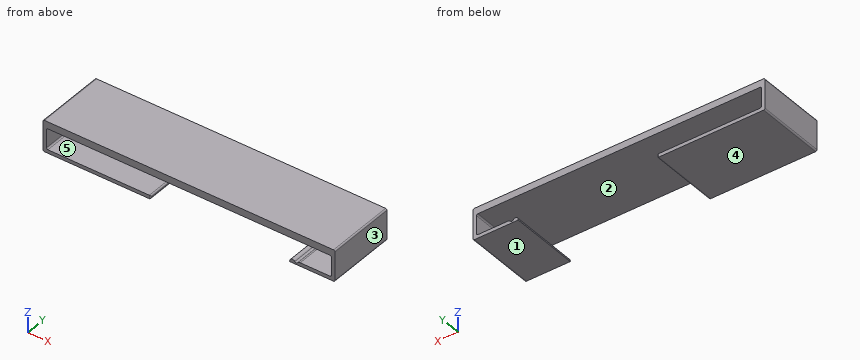
```python
from build123d import *

# Parameters (mm, degrees)
SKETCH1_W           = 15.5
SKETCH1_H           = 10
BOSS_EXTRUDE1_DEPTH = 0.5
SKETCH2_W           = 0.5
SKETCH2_H           = 10
BOSS_EXTRUDE2_DEPTH = 3
SKETCH3_W           = 42
SKETCH3_H           = 10
BOSS_EXTRUDE3_DEPTH = 1
SKETCH4_W           = 0.5
SKETCH4_H           = 10
BOSS_EXTRUDE4_DEPTH = 4.5
BOSS_EXTRUDE5_DEPTH = 10
FILLET1_R           = 0.2


with BuildPart() as part:
    # Sketch1 → Boss-Extrude1 (new body)
    with BuildSketch(Plane.XY):
        with Locations((-134.781169153, 115.619026916)):
            Rectangle(SKETCH1_W, SKETCH1_H)
    extrude(amount=BOSS_EXTRUDE1_DEPTH)

    # Sketch2 → Boss-Extrude2 (add)
    with BuildSketch(Plane.XY.offset(0.5)):
        with Locations((-142.281169153, 115.619026916)):
            Rectangle(SKETCH2_W, SKETCH2_H)
    extrude(amount=BOSS_EXTRUDE2_DEPTH)

    # Sketch3 → Boss-Extrude3 (add)
    with BuildSketch(Plane.XY.offset(3.5)):
        with Locations((-121.531169153, 115.619026916)):
            Rectangle(SKETCH3_W, SKETCH3_H)
    extrude(amount=BOSS_EXTRUDE3_DEPTH)

    # Sketch4 → Boss-Extrude4 (add)
    with BuildSketch(Plane.XY.offset(4.5)):
        with Locations((-100.781169153, 115.619026916)):
            Rectangle(SKETCH4_W, SKETCH4_H)
    extrude(amount=-BOSS_EXTRUDE4_DEPTH)

    # Sketch6 → Boss-Extrude5 (add)
    with BuildSketch(Plane(origin=(0, 110.619026916, 0), x_dir=(-1, 0, 0), z_dir=(0, -1, 0))):
        with BuildLine():
            Line((100.531169153, 0), (107.031169153, 0))
            Line((107.031169153, 0), (107.031169153, -0.1))
            ThreePointArc((107.031169153, -0.1), (106.754872908, -0.48039109), (106.307682248, -0.335279031))
            ThreePointArc((106.307682248, -0.335279031), (106.114215823, -0.2324803), (105.914058339, -0.321552283))
            ThreePointArc((105.914058339, -0.321552283), (105.742384515, -0.453197607), (105.531169153, -0.5))
            Line((105.531169153, -0.5), (100.531169153, -0.5))
            Line((100.531169153, -0.5), (100.531169153, 0))
        make_face()
    extrude(amount=-BOSS_EXTRUDE5_DEPTH)

    # Fillet1
    fillet1_edges = [part.edges().sort_by_distance(p)[0] for p in [
        (-127.031169153, 115.619026916, 0.5),
        (-142.031169153, 115.619026916, 0.5),
        (-142.031169153, 115.619026916, 3.5),
        (-142.531169153, 115.619026916, 4.5),
        (-100.531169153, 115.619026916, 4.5),
        (-100.531169153, 115.619026916, 0),
        (-101.031169153, 115.619026916, 3.5),
        (-127.031169153, 115.619026916, 0),
        (-142.531169153, 115.619026916, 0),
        (-101.031169153, 115.619026916, 0.5),
        (-127.031169153, 120.619026916, 0.25),
        (-127.031169153, 110.619026916, 0.25),
    ]]
    fillet(fillet1_edges, radius=FILLET1_R)


solid = part.part
```
Could you check a few things on this model? Use its own coordinates, in mm. Face numbers are marked on the shaded views. A direction names the side the tool comes from. Round coordinates to 2 decimals unless told otherwise and drop trailing zeros. Loops run counter-clockwise (first coordinate to the right, second up) from the corner with the lowest first, then second, coordinate; pieces in that order, holes last. Notation, with made-up numbers: (50, -32.75) - (92, -32.75) arc R34 ccw to (92, 6.25) - close; hole circle Ø10 at (58, 66.5). An arc over 180 degrees is marked (long way). Use CSV: the item, a comma, the result in double quotes.
Item 1: If we section it at B-B on x = -137: List the corners of the cut face in (y, z) for me.
Here are the results:
outline,"(110.62, 0) - (120.62, 0) - (120.62, 0.5) - (110.62, 0.5) - close; (110.62, 3.5) - (120.62, 3.5) - (120.62, 4.5) - (110.62, 4.5) - close"
Item 2: If we section it at D-D on x = -118: List the corners of the cut face in (y, z) for me.
Here are the results:
outline,"(110.62, 3.5) - (120.62, 3.5) - (120.62, 4.5) - (110.62, 4.5) - close"
Item 3: If we mould it in two halves opening along Z, with no side actions, what happens to the marked faces 3, 4 and 5? For each: pulls with the +Z half, pulls with the -Z half, needs draft (parallel to the pull), parting line crosses it, or undercut.
Here are the results:
face 3,"needs draft"
face 4,"pulls with the -Z half"
face 5,"undercut"
Item 4: If we section it at C-C on y = 113.5: List the corners of the cut face in (x, z) for me, then the cut area to 3 significant figures.
Here are the results:
outline,"(-142.53, 0.2) arc R0.2 ccw to (-142.33, 0) - (-127.23, 0) arc R0.2 ccw to (-127.03, 0.2) - (-127.03, 0.3) arc R0.2 ccw to (-127.23, 0.5) - (-141.83, 0.5) arc R0.2 cw to (-142.03, 0.7) - (-142.03, 3.3) arc R0.2 cw to (-141.83, 3.5) - (-101.23, 3.5) arc R0.2 cw to (-101.03, 3.3) - (-101.03, 0.7) arc R0.2 cw to (-101.23, 0.5) - (-105.53, 0.5) arc R0.5 ccw to (-105.91, 0.32) arc R0.25 cw to (-106.31, 0.34) arc R0.4 ccw to (-107.03, 0.1) - (-107.03, 0) - (-100.73, 0) arc R0.2 ccw to (-100.53, 0.2) - (-100.53, 4.3) arc R0.2 ccw to (-100.73, 4.5) - (-142.33, 4.5) arc R0.2 ccw to (-142.53, 4.3) - close"
area,"55.8 mm²"
Item 5: For the marked faces 1 and 2, which set-ups out of +Z, -Z, +X, -X, +Y, -Y let a thin tool reach every point of the face, with its end or its side?
Here are the results:
face 1,"-Z, +X, -X, +Y, -Y"
face 2,"+Y, -Y"
Item 6: If we section it at A-A on z = 2.45: List the corners of the cut face in (x, y) for me.
Here are the results:
outline,"(-142.53, 110.62) - (-142.03, 110.62) - (-142.03, 120.62) - (-142.53, 120.62) - close; (-101.03, 110.62) - (-100.53, 110.62) - (-100.53, 120.62) - (-101.03, 120.62) - close"
Item 7: I need wall thicknesses on L1, parallel to Z at x = -138, y = 112.25; L2, parallel to X at y = 115.5, z = 2.35; L3, parallel to X at y = 117, z = 0.4. Which ranges of each line are inside material? Lowest first, please. Write a range as [from, to].
Here are the results:
L1,"z = [0, 0.5], [3.5, 4.5]"
L2,"x = [-142.53, -142.03], [-101.03, -100.53]"
L3,"x = [-142.53, -127.06], [-106.9, -106.37], [-105.83, -100.53]"
